Drawing for the job (mm, zero at the part's lowest x, y, z). Coordinates: 2 decimals unless noted, no trailing zeros. Order: outer loops, then holes, each group sorted by start corner. A loop starts at its lowest first (then second) coordinate and runs counter-clockwise, first axis right, second up.
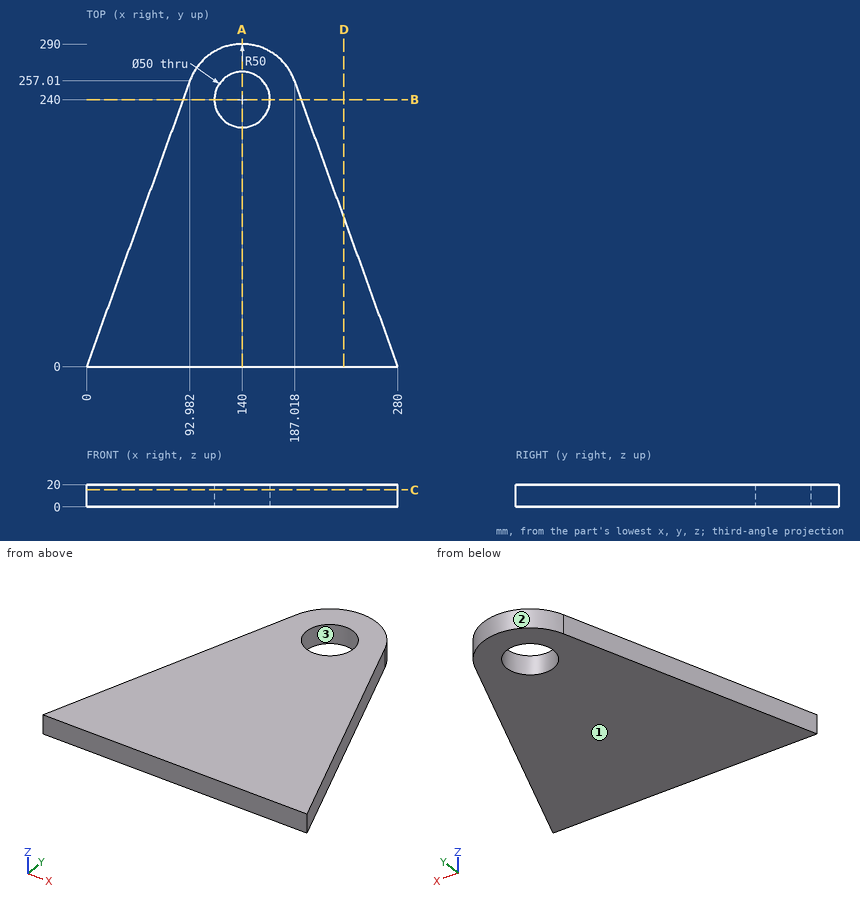
1) Slice it at A-A (x = 140). List the corners of the cut face in (y, z), plus the area to 3 significant figures.
2) Pin check, flat tips, straight feed: P1, Ø1, axis at y = 45.5, z = 14.5, coming from the -X side; P2, Ø1, axis at y = 177, z = 5.5, coming from the -X side (1 decimal); P3, Ø8, axis at y = 235.5, z = 16.5, coming from the -X side. Stop position of each tip, or through.
3) Two-plate mould, pull along Y, no slides. Class the marked faces 1, 2 and 3: released by +Y, released by -Y, zero draft, split by the parting line, or undercut.
4) Drill centre lines: probe 1 along Y at (x, z) = (119, 6.5) (1 decimal); probe 2 along X at (y, z) = (233, 18.5) (1 decimal); probe 3 along Y at (x, z) = (114, 10). Where is each one in solid material? Low to high.
5) Slice it at C-C (z = 15.25). List the corners of the cut face in (x, y), plus the area to 3 significant figures.
6) Slice it at B-B (y = 240). List the corners of the cut face in (x, z).
7) Slice it at D-D (x = 231.5). List the corners of the cut face in (y, z).
Worked out:
1. outline: (0, 0) - (215, 0) - (215, 20) - (0, 20) - close; (265, 0) - (290, 0) - (290, 20) - (265, 20) - close
1. area: 4,800 mm2
2. P1: stops at x = 16.28
2. P2: stops at x = 63.9
2. P3: stops at x = 83.75
3. face 1: zero draft
3. face 2: released by +Y
3. face 3: undercut
4. probe 1: y = 0 to 226.4, 253.6 to 285.4
4. probe 2: x = 84.3 to 116, 164 to 195.7
4. probe 3: y = 0 to 282.71
5. outline: (0, 0) - (280, 0) - (187.02, 257.01) arc R50 ccw to (92.98, 257.01) - close; hole circle Ø50 at (140, 240)
5. area: 48,400 mm2
6. outline: (86.83, 0) - (115, 0) - (115, 20) - (86.83, 20) - close; (165, 0) - (193.17, 0) - (193.17, 20) - (165, 20) - close
7. outline: (0, 0) - (134.06, 0) - (134.06, 20) - (0, 20) - close
